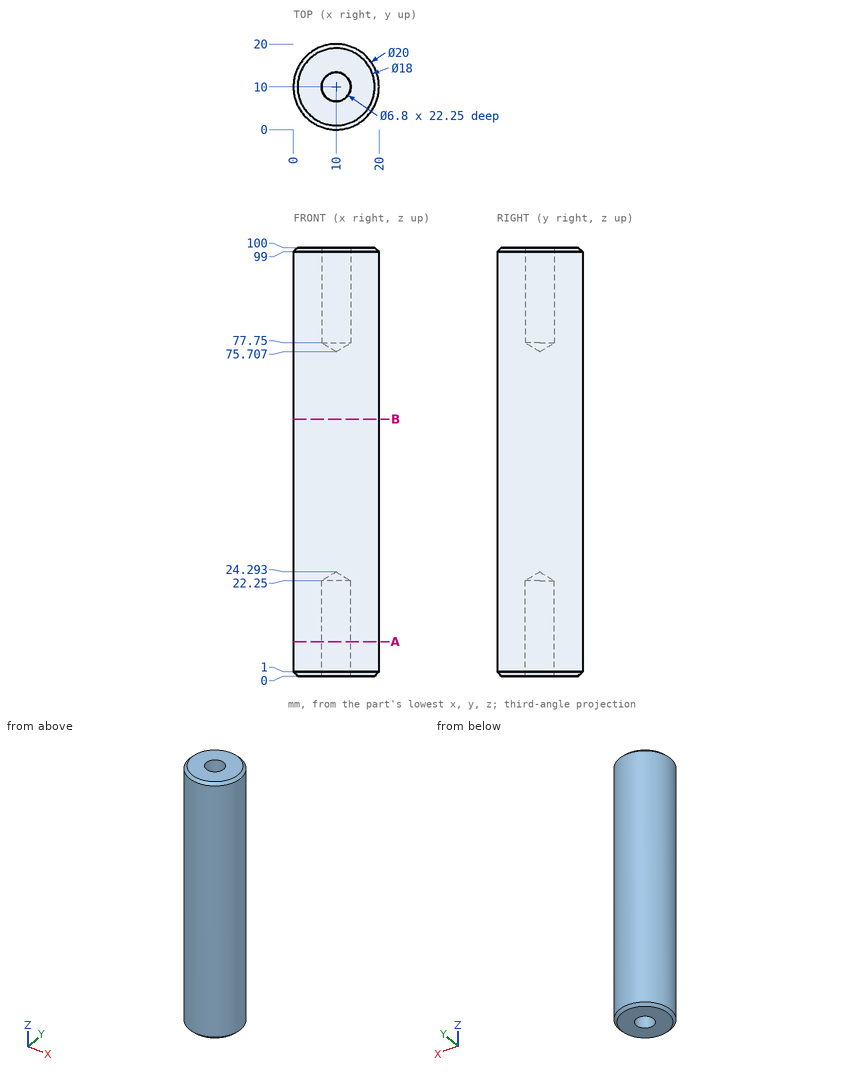
Check sheet for the drawn part. Datum: minimum x, y, z corner. Units: mm. Give positions to 0.01 mm unless a question says otherwise; leave off trailing zeros. Loops run counter-clockwise (first coordinate to the right, second up) from the corner with the lowest first, then second, coordinate; pieces in that order, holes last. Notation, with made-up numbers: M 9,89 L 60,89 A11 ccw 60,94 Z; hole C 8,55.5 d6. An arc over 180 degrees is marked long. Answer as CSV lines item,"result".
Item 1: Depth check by flat-ended pin: pin 1 Ø1.5 at (x, z) = (7.5, 13) entering from -Y; pin 2 Ø1 at (y, z) = (15.5, 18) entering from +X; pin 3 Ø4 at (x, y) = (10, 10) entering from +Z. Enter the tip coordinate at first touch or a pass-through.
Reply:
pin 1,"y = 0.15"
pin 2,"x = 18.66"
pin 3,"z = 76.91"
Item 2: Sectioned sample at B-B, the plane z = 60. Enter the section's corners in (x, y).
Reply:
outline,"C 10,10 d20"
Item 3: Scan lines: L1, parallel to Y at x = 10, z = 86; L2, parallel to Y at x = 9.75, z = 28.5; L3, parallel to Y at x = 3, z = 5. Record each from-to range of solid material in increasing order.
Reply:
L1,"0 to 6.6, 13.4 to 20"
L2,"0 to 20"
L3,"2.86 to 17.14"
Item 4: Sectioned sample at A-A, the plane z = 8. Enter the section's corners in (x, y), then the cut area to 3 significant figures.
Reply:
outline,"C 10,10 d20; hole C 10,10 d6.8"
area,"278 mm^2"
